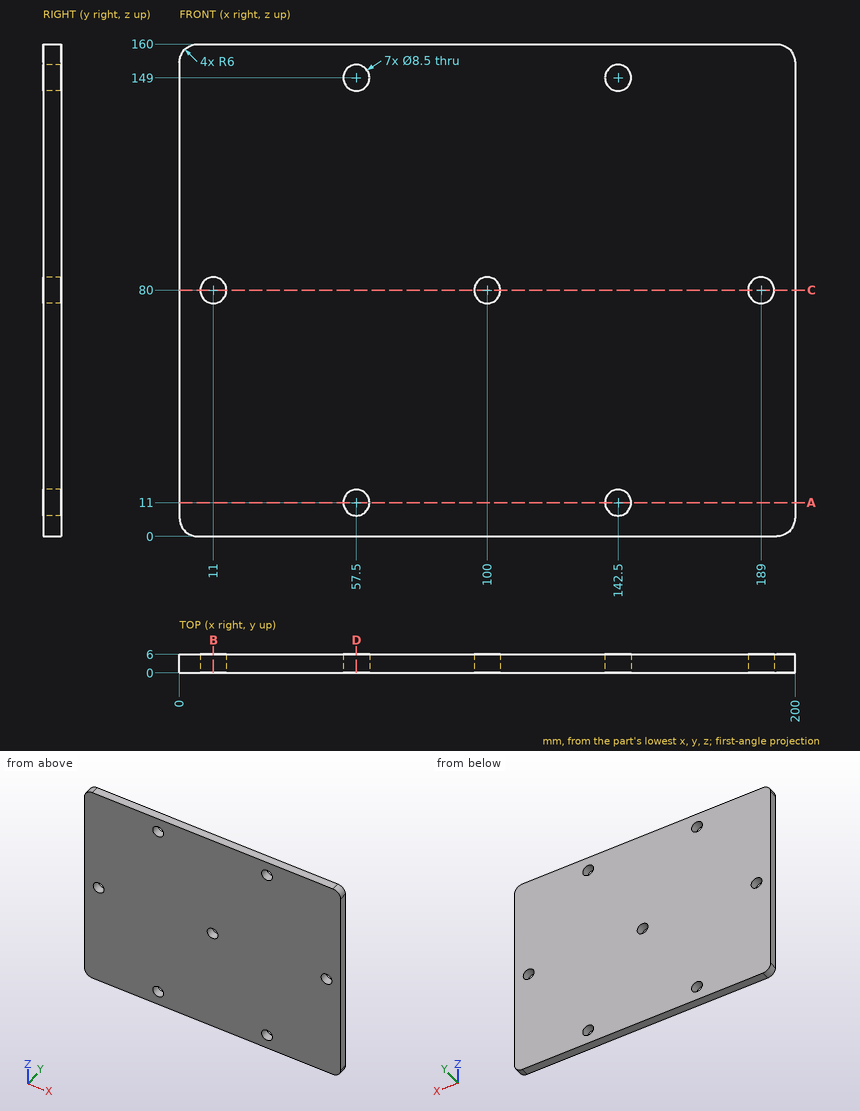
Geometry: see drawing. Coordinates: mm, zero at the bounding-box minimum. Coordinates: 2 decimals unless noted, no trailing zeros. Order: outer loops, then holes, each group sorted by start corner. A loop starts at its lowest first (then second) coordinate and runs counter-clockwise, first axis right, second up. Notation, with made-up numbers: (10.25, 47.25) -> (51.25, 47.25) arc R12 ccw to (51.25, 58.25) -> close; hole circle Ø6 at (47, -31.5). An arc over 180 degrees is marked (long way). Write each question's results on one line, items separated by ' | '. Start each with the question number.
1) Material intervals for line 1 along Z through (x, y) = (57.5, 2.45); line 2 along X through (y, z) = (2.85, 80); line 3 along X through (y, z) = (3.8, 11), sorted ascending.
2) Cut plane B-B, the plane x = 11. Output: boundary loops of the cut face in (y, z).
3) Cut plane D-D, the plane x = 57.5. Output: boundary loops of the cut face in (y, z).
4) Cut plane C-C, the plane z = 80. Output: boundary loops of the cut face in (x, y).
5) Cut plane A-A, the plane z = 11. Output: boundary loops of the cut face in (x, y), and give its area (3 significant figures).
Checks:
1) line 1: 0 to 6.75, 15.25 to 144.75, 153.25 to 160 | line 2: 0 to 6.75, 15.25 to 95.75, 104.25 to 184.75, 193.25 to 200 | line 3: 0 to 53.25, 61.75 to 138.25, 146.75 to 200
2) outline: (0, 0) -> (6, 0) -> (6, 75.75) -> (0, 75.75) -> close; (0, 84.25) -> (6, 84.25) -> (6, 160) -> (0, 160) -> close
3) outline: (0, 0) -> (6, 0) -> (6, 6.75) -> (0, 6.75) -> close; (0, 15.25) -> (6, 15.25) -> (6, 144.75) -> (0, 144.75) -> close; (0, 153.25) -> (6, 153.25) -> (6, 160) -> (0, 160) -> close
4) outline: (0, 0) -> (6.75, 0) -> (6.75, 6) -> (0, 6) -> close; (15.25, 0) -> (95.75, 0) -> (95.75, 6) -> (15.25, 6) -> close; (104.25, 0) -> (184.75, 0) -> (184.75, 6) -> (104.25, 6) -> close; (193.25, 0) -> (200, 0) -> (200, 6) -> (193.25, 6) -> close
5) outline: (0, 0) -> (53.25, 0) -> (53.25, 6) -> (0, 6) -> close; (61.75, 0) -> (138.25, 0) -> (138.25, 6) -> (61.75, 6) -> close; (146.75, 0) -> (200, 0) -> (200, 6) -> (146.75, 6) -> close | area: 1,100 mm^2
